For this review, take the finished solid that the model builds, in its own axes (mm). Face numbers are marked on the shaded views. A direction names the side the tool comes from. Coordinates: 2 decimals unless noted, no trailing zeros. Write each loop counter-clockwise with the first axis right and the second up, starting at its lowest first coordinate (ties: lowest second). Pieces come first, ordered by that corner, then holes.
1) To check wall thickness, follow line 1 along Y through (x, z) = (17, 25); line 2 along Z through (x, y) = (10, 61.25); line 3 along Z through (x, y) = (5.5, 45). State the ranges of each line that lie inside material, in increasing order.
2) Mouldability with a two-part tool opening along Y and no side actions: class the marked faces 3, 4 and 5 as pulls with the +Y half, pulls with the -Y half, needs draft (parallel to the pull), parting line crosses it, or undercut.
3) We need section D-D on y = -5. Write out the cut boundary in (x, z) (3 decimals), then the cut area to 3 significant figures.
4) We need section C-C on x = 17.75. Write out the cut boundary in (y, z).
5) We need section A-A on z = -4.5. Write out the cut boundary in (x, y).
6) Insertion check: P1, Ø3, axis at x = 10, z = 30, coming from the -Y side; P2, Ø11.5, axis at y = -5, z = 25, coming from the +X side; P3, Ø11.5, axis at y = 45, z = 25, coming from the -X side (3 decimals). Each pin has a flat end and moves straight along its axis. Give the tip position at first contact, or say it passes through.
7) We need section B-B on y = 27.5. Write out the cut boundary in (x, z), then the cut area to 3 significant figures.
8) For the marked faces 1 and 2, list the 3-axis set-ups (+Z, -Z, +X, -X, +Y, -Y) from which the entire face can be reached by the end or side of a thin tool; tool diameter is ignored.
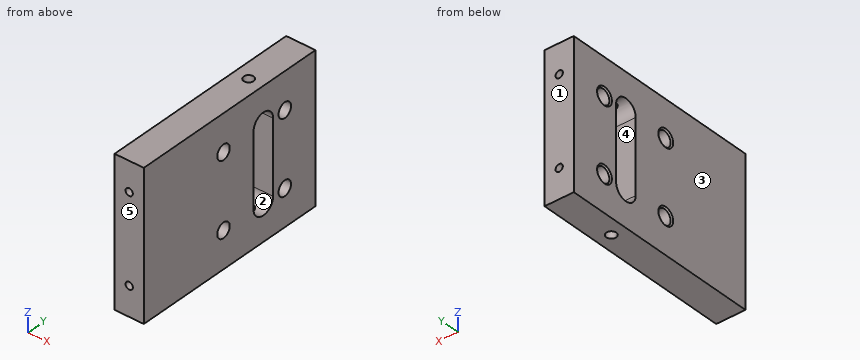
from build123d import *

# Parameters (mm, degrees)
SKETCH_1_W                    = 100
SKETCH_1_H                    = 140
EXTRUDE_1_DEPTH               = 20
HOLE_WIZARD_M6_1_D            = 5
HOLE_WIZARD_M6_1_DEPTH        = 15
HOLE_WIZARD_M6_1_TIP          = 1.502151548
CUT_EXTRUDE_1_DEPTH           = 89.317608663
HOLE_WIZARD_M8_1_D            = 6.8
HOLE_WIZARD_M12_1_D           = 10.2
HOLE_WIZARD_M12_1_CSINK_D     = 12.05
HOLE_WIZARD_M12_1_CSINK_ANGLE = 90
HOLE_WIZARD_M6_2_D            = 5
HOLE_WIZARD_M6_2_DEPTH        = 15
HOLE_WIZARD_M6_2_TIP          = 1.502151548


with BuildPart() as part:
    # 草图1 → 凸台-拉伸1 (new body)
    with BuildSketch(Plane(origin=(0, 0, 0), x_dir=(0, 0, -1), z_dir=(1, 0, 0))):
        Rectangle(SKETCH_1_W, SKETCH_1_H)
    extrude(amount=EXTRUDE_1_DEPTH)

    # M6 螺纹孔1
    with Locations(Plane(origin=(0, -70, 0), x_dir=(-1, 0, 0), z_dir=(0, -1, 0))):
        with Locations((-10, 30), (-10, -30)):
            Hole(HOLE_WIZARD_M6_1_D / 2, depth=HOLE_WIZARD_M6_1_DEPTH)
            with Locations((0, 0, -(HOLE_WIZARD_M6_1_DEPTH + HOLE_WIZARD_M6_1_TIP / 2))):  # 118° drill point
                Cone(0, HOLE_WIZARD_M6_1_D / 2, HOLE_WIZARD_M6_1_TIP, mode=Mode.SUBTRACT)

    # 草图4 → 切除-拉伸1 (cut, through all)
    with BuildSketch(Plane.ZY):
        with BuildLine():
            Line((-25, 35.5), (25, 35.5))
            ThreePointArc((25, 35.5), (33, 27.5), (25, 19.5))
            Line((25, 19.5), (-25, 19.5))
            ThreePointArc((-25, 19.5), (-33, 27.5), (-25, 35.5))
        make_face()
    extrude(amount=-CUT_EXTRUDE_1_DEPTH, mode=Mode.SUBTRACT)

    # M8 螺纹孔1 (through all)
    with Locations(Plane.XY.offset(50)):
        with Locations((10, 27.5)):
            Hole(HOLE_WIZARD_M8_1_D / 2)

    # M12 螺纹孔1 (through all)
    with Locations(Plane.ZY):
        with Locations((-25, 45), (25, 45), (-25, -5), (25, -5)):
            CounterSinkHole(HOLE_WIZARD_M12_1_D / 2, HOLE_WIZARD_M12_1_CSINK_D / 2, counter_sink_angle=HOLE_WIZARD_M12_1_CSINK_ANGLE)

    # M6 螺纹孔2
    with Locations(Plane(origin=(0, 70, 0), x_dir=(1, 0, 0), z_dir=(0, 1, 0))):
        with Locations((10, 30), (10, -30)):
            Hole(HOLE_WIZARD_M6_2_D / 2, depth=HOLE_WIZARD_M6_2_DEPTH)
            with Locations((0, 0, -(HOLE_WIZARD_M6_2_DEPTH + HOLE_WIZARD_M6_2_TIP / 2))):  # 118° drill point
                Cone(0, HOLE_WIZARD_M6_2_D / 2, HOLE_WIZARD_M6_2_TIP, mode=Mode.SUBTRACT)


solid = part.part
Result:
1. line 1: y = -70 to -10.1, 0.1 to 19.5, 35.5 to 39.9, 50.1 to 70
1. line 2: z = -50 to -32.5, -27.5 to 27.5, 32.5 to 50
1. line 3: z = -50 to -30.1, -19.9 to 19.9, 30.1 to 50
2. face 3: needs draft
2. face 4: undercut
2. face 5: pulls with the -Y half
3. outline: (0, -50) - (20, -50) - (20, -30.1) - (0.925, -30.1) - (0, -31.025) - close; (0, -18.975) - (0.925, -19.9) - (20, -19.9) - (20, 19.9) - (0.925, 19.9) - (0, 18.975) - close; (0, 31.025) - (0.925, 30.1) - (20, 30.1) - (20, 50) - (0, 50) - close
3. area: 1,590 mm2
4. outline: (-70, -50) - (70, -50) - (70, 50) - (-70, 50) - close; hole circle Ø10.2 at (-5, -25); hole circle Ø10.2 at (-5, 25); hole (19.5, -25) arc R8 ccw to (35.5, -25) - (35.5, 25) arc R8 ccw to (19.5, 25) - close; hole circle Ø10.2 at (45, -25); hole circle Ø10.2 at (45, 25)
5. outline: (0, -70) - (20, -70) - (20, 19.5) - (0, 19.5) - close; (0, 35.5) - (20, 35.5) - (20, 70) - (0, 70) - close
6. P1: stops at y = -54.4
6. P2: stops at x = 20
6. P3: stops at x = 0.275
7. outline: (0, -50) - (6.6, -50) - (6.6, -33) - (0, -33) - close; (0, 33) - (6.6, 33) - (6.6, 50) - (0, 50) - close; (13.4, -50) - (20, -50) - (20, -33) - (13.4, -33) - close; (13.4, 33) - (20, 33) - (20, 50) - (13.4, 50) - close
7. area: 449 mm2
8. face 1: +Z, -Z, +X, -X, +Y
8. face 2: +X, -X
